Verification items for this drawing (mm, ordinates from the low corner). Round coordinates to 2 decimals unless told otherwise and drop trailing zeros. Loops run counter-clockwise (first coordinate to the right, second up) from the corner with the lowest first, then second, coordinate; pieces in that order, holes last. Notation, with made-up numbers: (-2.5, 13.25) - (27.5, 13.25) arc R14 ccw to (27.5, 35.25) - close; hole circle Ø6 at (6.5, -29). An arc over 180 degrees is marked (long way). Answer in a Markdown table with one row per item. Add a question column.
(1) Cross-section at C-C on x = 47. Enter the section's corners in (y, z), then the cut area to 3 significant figures.
(2) Thickness scan on line 1 along X through (y, z) = (54.5, 1.6); line 2 along Y through (x, z) = (41, 0.9); line 3 along Y through (x, z) = (114, 3.35). Record the ranges inside material, lowest first.
(3) Cross-section at B-B on z = 1. Enter the section's corners in (x, y).
(4) Cross-section at A-A on y = 86. Enter the section's corners in (x, z), then the cut area to 3 significant figures.
(5) Cross-section at D-D on x = 103.5. Enter the section's corners in (y, z), then the cut area to 3 significant figures.
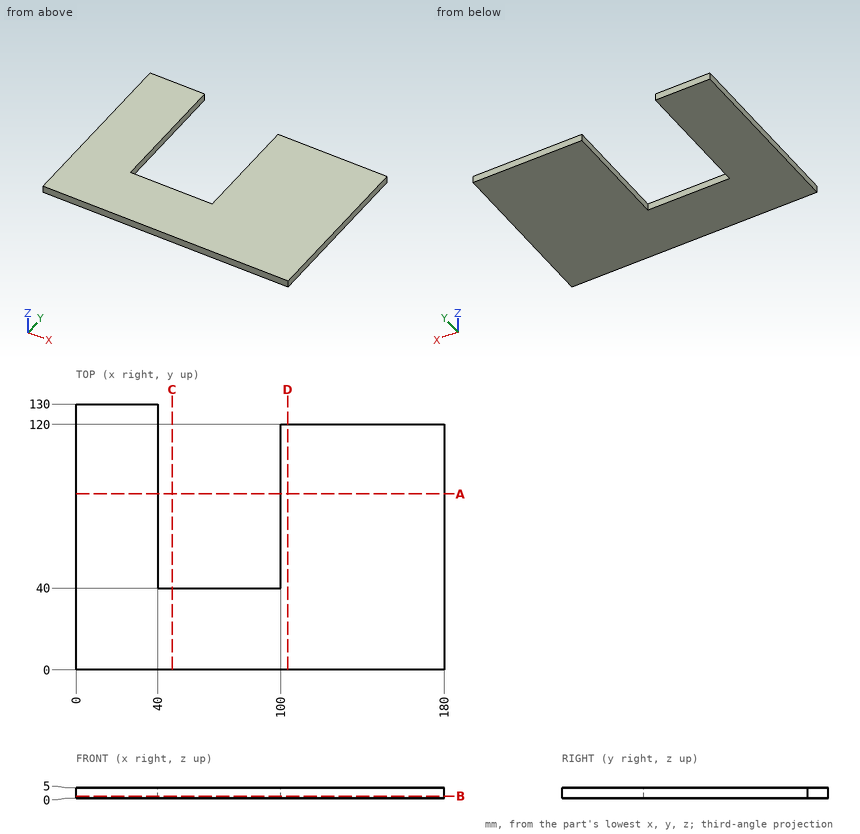
Answers:
| question | item | result |
|---|---|---|
| 1 | outline | (0, 0) - (40, 0) - (40, 5) - (0, 5) - close |
| 1 | area | 200 mm^2 |
| 2 | line 1 | x = 0 to 40, 100 to 180 |
| 2 | line 2 | y = 0 to 40 |
| 2 | line 3 | y = 0 to 120 |
| 3 | outline | (0, 0) - (180, 0) - (180, 120) - (100, 120) - (100, 40) - (40, 40) - (40, 130) - (0, 130) - close |
| 4 | outline | (0, 0) - (40, 0) - (40, 5) - (0, 5) - close; (100, 0) - (180, 0) - (180, 5) - (100, 5) - close |
| 4 | area | 600 mm^2 |
| 5 | outline | (0, 0) - (120, 0) - (120, 5) - (0, 5) - close |
| 5 | area | 600 mm^2 |
